The model under review builds one solid part; all positions refer to its coordinate system, in mm. Face numbers are marked on the shaded views. A direction names the side the tool comes from. Round coordinates to 2 decimals unless told otherwise and drop trailing zeros. Loops run counter-clockwise (first coordinate to the right, second up) from the corner with the lowest first, then second, coordinate; pieces in that order, holes last. Notation, with made-up numbers: (48, 54) -> (69, 54) arc R11 ccw to (69, 58) -> close; hole circle Ø7 at (86, 44.25). An arc over 180 degrees is marked (long way). Write each question's results on one line, items separated by ' | '. Start each with the question number.
Item 1: Mouldability with a two-part tool opening along Y and no side actions: class the marked faces 1, 2, 3 and 4 as pulls with the +Y half, pulls with the -Y half, needs draft (parallel to the pull), parting line crosses it, or undercut.
Item 2: We need section C-C (z = 2.25). Give the boundary of the cut face in (x, y).
Item 3: Clearance check with flat-ended pins moving along their axes: pin 1 Ø4 at (x, z) = (8.5, 10) entering from +Y; pin 2 Ø1 at (x, z) = (2.5, 7.5) entering from -Y; pin 3 Ø1.5 at (x, y) = (-1, -0.5) entering from +Z. State where each tip first meets the part, or that it passes through.
Item 4: For L1, parallel to Y at x = -0.5, z = 10.25; L2, parallel to Z at x = -1, y = 12; L3, parallel to Y at x = 3.25, z = 16, list the stretches that pass through material, from the lowest coordinate up. Write a range as from..to.
Item 5: Tool access review of the marked faces 5 and 6: name each direction out of +Z, -Z, +X, -X, +Y, -Y from which nothing blocks a thin tool from reaching the whole face with its end or side.
Item 6: We need section B-B (y = 5.5). Give the boundary of the cut face in (x, z), and give its area (3 significant figures).
Item 7: We need section A-A (z = 18.25). Give the boundary of the cut face in (x, y).
from build123d import *

# Parameters (mm, degrees)
BOSS_EXTRUDE1_DEPTH = 22
SKETCH2_W           = 22
SKETCH2_H           = 25
CUT_EXTRUDE1_DEPTH  = 18
CHAMFER1_SIZE       = 0.5


with BuildPart() as part:
    # Sketch1 → Boss-Extrude1 (new body)
    with BuildSketch(Plane.XY):
        with BuildLine():
            Line((11, -15.491933385), (11, 15.491933385))
            ThreePointArc((11, 15.491933385), (0, 19), (-11, 15.491933385))
            Line((-11, 15.491933385), (-11, -15.491933385))
            ThreePointArc((-11, -15.491933385), (0, -19), (11, -15.491933385))
        make_face()
    extrude(amount=BOSS_EXTRUDE1_DEPTH)

    # Sketch2 → Cut-Extrude1 (cut)
    with BuildSketch(Plane.XY.offset(22)):
        Rectangle(SKETCH2_W, SKETCH2_H)
    extrude(amount=-CUT_EXTRUDE1_DEPTH, mode=Mode.SUBTRACT)

    # Chamfer1
    chamfer1_edges = [part.edges().sort_by_distance(p)[0] for p in [
        (0, 19, 22),
        (0, -19, 22),
        (0, 19, 0),
        (0, -19, 0),
    ]]
    chamfer(chamfer1_edges, length=CHAMFER1_SIZE)


solid = part.part
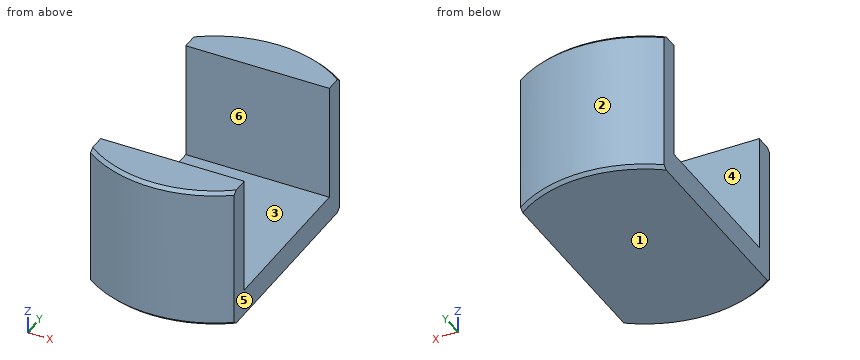
Here are the results:
1) face 1: needs draft | face 2: pulls with the +Y half | face 3: undercut | face 4: undercut
2) outline: (-11, -15.49) arc R19 ccw to (11, -15.49) -> (11, 15.49) arc R19 ccw to (-11, 15.49) -> close
3) pin 1: stops at y = 17.85 | pin 2: stops at y = -18.89 | pin 3: stops at z = 4
4) L1: y = -18.99..-12.5, 12.5..18.99 | L2: z = 0..4 | L3: y = -18.72..-12.5, 12.5..18.72
5) face 5: +Z, -Z, +X, +Y, -Y | face 6: +Z, +X, -X
6) outline: (-11, 0) -> (11, 0) -> (11, 4) -> (-11, 4) -> close | area: 88.0 mm2
7) outline: (-11, -15.49) arc R19 ccw to (11, -15.49) -> (11, -12.5) -> (-11, -12.5) -> close; (-11, 12.5) -> (11, 12.5) -> (11, 15.49) arc R19 ccw to (-11, 15.49) -> close
